Build history of the part. All positions in model axes, mm. Face numbers are marked on the shaded views. A direction names the side the tool comes from. Round coordinates to 2 decimals unless told otherwise and drop trailing zeros. Write each loop counter-clockwise with the first axis right and the second up, starting at its lowest first coordinate (ties: lowest second). Pieces come first, ordered by that corner, then holes. Notation, with made-up numbers: M 88,44.25 L 99,44.25 A31 ccw 99,80.25 Z; hole C 11.5,75.25 d3. An arc over 180 degrees is marked long. Use a Markdown table: item, result.
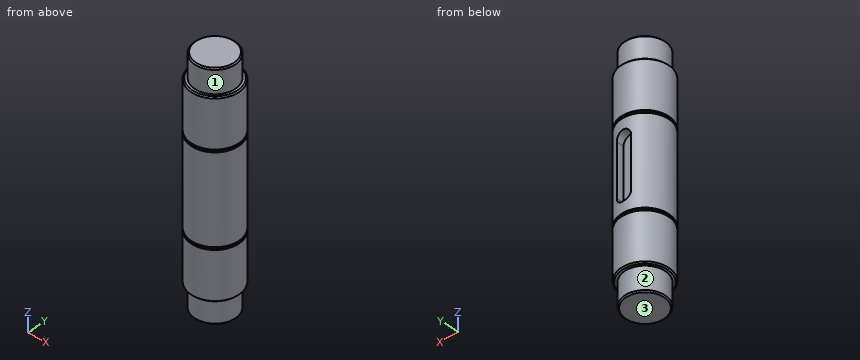
from build123d import *

# Parameters (mm, degrees)
SKETCH_1_R          = 10
EXTRUDE_1_DEPTH     = 40
SKETCH_2_R          = 8.5
EXTRUDE_2_DEPTH     = 10
CUT_EXTRUDE_START   = 1.1
SKETCH_4_R          = 10
SKETCH_4_R_2        = 9.5
CUT_EXTRUDE_1_DEPTH = 1.1
CHAMFER_1_SIZE      = 0.5
CUT_EXTRUDE_2_DEPTH = 3.5


with BuildPart() as part:
    # 草图1 → 凸台-拉伸1 (new, symmetric)
    with BuildSketch(Plane.XY):
        Circle(SKETCH_1_R)
    extrude(amount=EXTRUDE_1_DEPTH, both=True)

    # 草图2 → 凸台-拉伸2 (add)
    with BuildSketch(Plane.XY.offset(40)):
        Circle(SKETCH_2_R)
    extrude_2 = extrude(amount=EXTRUDE_2_DEPTH)

    # 草图4 → 切除-拉伸1 (cut)
    with BuildSketch(Plane.XY.offset(18.5).offset(CUT_EXTRUDE_START)):
        Circle(SKETCH_4_R)
        Circle(SKETCH_4_R_2, mode=Mode.SUBTRACT)
    cut_extrude_1 = extrude(amount=-CUT_EXTRUDE_1_DEPTH, mode=Mode.SUBTRACT)

    # 镜向1: 凸台-拉伸2, 切除-拉伸1 across plane
    add(extrude_2.mirror(Plane.XY))
    add(cut_extrude_1.mirror(Plane.XY), mode=Mode.SUBTRACT)

    # 倒角1
    chamfer_1_edges = [part.edges().sort_by_distance(p)[0] for p in [
        (-8.5, 0, -50),
        (-10, 0, -40),
        (-10, 0, 40),
        (-8.5, 0, 50),
    ]]
    chamfer(chamfer_1_edges, length=CHAMFER_1_SIZE)

    # 草图5 → 切除-拉伸2 (cut)
    with BuildSketch(Plane(origin=(0, 10, 0), x_dir=(1, 0, 0), z_dir=(0, 1, 0))):
        with BuildLine():
            Line((3, 11), (3, -11))
            ThreePointArc((3, -11), (0, -14), (-3, -11))
            Line((-3, -11), (-3, 11))
            ThreePointArc((-3, 11), (0, 14), (3, 11))
        make_face()
    extrude(amount=-CUT_EXTRUDE_2_DEPTH, mode=Mode.SUBTRACT)


solid = part.part
Q1. Drill centre lines: L1, parallel to Z at x = 7.5, y = -6; L2, parallel to Z at x = 2.5, y = -8.5; L3, parallel to Y at x = 0.5, z = 45.5. Where is each one in solid material? Low to high.
Response values:
| item | result |
|---|---|
| L1 | z = -39.9 to -19.6, -18.5 to 18.5, 19.6 to 39.9 |
| L2 | z = -40 to 40 |
| L3 | y = -8.49 to 8.49 |
Q2. Drop flat-ended pins along their axis: P1, Ø1.5, axis at x = -5.5, z = 28, coming from the +Y side; P2, Ø8, axis at y = -6, z = 12, coming from the -X side; P3, Ø1.5, axis at y = 8, z = 3.5, coming from the +X side. Give the stop position or say it passes through.
Response values:
| item | result |
|---|---|
| P1 | stops at y = 8.8 |
| P2 | stops at x = -9.8 |
| P3 | stops at x = 6.89 |
Q3. Cut at A-A on z = -29. Give the cut face in (x, y).
Response values:
| item | result |
|---|---|
| outline | C 0,0 d20 |
Q4. Which spindle directions (+Z, -Z, +X, -X, +Y, -Y) get a long thin tool onto all of the face, cutting with end or side? Do the marked faces 1, 2 and 3. Say none if no direction does.
Response values:
| item | result |
|---|---|
| face 1 | +Z |
| face 2 | -Z |
| face 3 | -Z, +X, -X, +Y, -Y |
